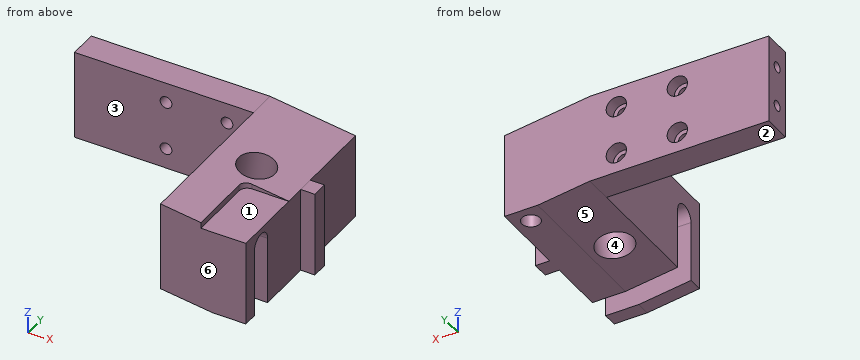
from build123d import *

# Parameters (mm, degrees)
EXTRUDE_1_DEPTH     = 23.69
CUT_EXTRUDE_1_REACH = 50.333
SKETCH_2_W          = 44
SKETCH_2_H          = 39
CUT_EXTRUDE_2_REACH = 75.348
CUT_EXTRUDE_3_DEPTH = 63.115721705
CUT_EXTRUDE_4_DEPTH = 2.79
CUT_EXTRUDE_5_REACH = 53.075
SKETCH_7_R          = 4.5
SKETCH_8_R          = 1.25
CUT_EXTRUDE_6_DEPTH = 8.5
SKETCH_10_R         = 1.45
CUT_EXTRUDE_7_DEPTH = 63.115721705
SKETCH_11_R         = 2.5
CUT_EXTRUDE_8_DEPTH = 3
SKETCH_12_R         = 2.25
CUT_EXTRUDE_9_DEPTH = 6


with BuildPart() as part:
    # 草图1 → 凸台-拉伸1 (new body)
    with BuildSketch(Plane.XY):
        Polygon((30.632183908, 5.365900383), (34.132183908, 5.365900383), (34.132183908, 1.365900383), (30.632183908, 1.365900383), (30.632183908, -21.634099617), (-34.367816092, -21.634099617), (-34.367816092, 24.365900383), (30.632183908, 24.365900383), align=None)
    extrude(amount=EXTRUDE_1_DEPTH)

    # 草图2 → 切除-拉伸1 (cut, up to next)
    with BuildSketch(Plane(origin=(0, 0, 0), x_dir=(-1, 0, 0), z_dir=(0, 0, -1)), mode=Mode.PRIVATE) as cut_extrude_1_sk1:
        with Locations((12.367816092, -2.134099617)):
            Rectangle(SKETCH_2_W, SKETCH_2_H)
    cut_extrude_1_tool1 = extrude(cut_extrude_1_sk1.sketch, amount=-CUT_EXTRUDE_1_REACH, mode=Mode.PRIVATE) & part.part
    add(cut_extrude_1_tool1.solids().sort_by_distance((-12.367816, -2.1341, 0))[0], mode=Mode.SUBTRACT)

    # 草图3 → 切除-拉伸2 (cut, up to next)
    with BuildSketch(Plane(origin=(30.632183908, 0, 0), x_dir=(0, 0, -1), z_dir=(1, 0, 0)), mode=Mode.PRIVATE) as cut_extrude_2_sk1:
        with BuildLine():
            Line((0, -18.084546462), (0, -12.484546462))
            Line((0, -12.484546462), (-16.69, -12.484546462))
            ThreePointArc((-16.69, -12.484546462), (-19.49, -15.284546462), (-16.69, -18.084546462))
            Line((-16.69, -18.084546462), (0, -18.084546462))
        make_face()
    cut_extrude_2_tool1 = extrude(cut_extrude_2_sk1.sketch, amount=-CUT_EXTRUDE_2_REACH, mode=Mode.PRIVATE) & part.part
    add(cut_extrude_2_tool1.solids().sort_by_distance((30.632184, -15.284546, 9.454896))[0], mode=Mode.SUBTRACT)

    # 草图4 → 切除-拉伸3 (cut, through all)
    with BuildSketch(Plane(origin=(0, 24.365900383, 0), x_dir=(1, 0, 0), z_dir=(0, 1, 0))):
        Polygon((9.632183908, -23.69), (34.132183908, -23.69), (34.132183908, -20.93), (30.632183908, -20.93), align=None)
        Polygon((-34.367816092, -1.69), (-34.367816092, 0), (22.482183908, 0), (9.632183908, -1.69), align=None)
    extrude(amount=-CUT_EXTRUDE_3_DEPTH, mode=Mode.SUBTRACT)

    # 草图5 → 切除-拉伸4 (cut)
    with BuildSketch(Plane.XY.offset(23.69)):
        with BuildLine():
            Line((30.632183908, -21.634099617), (19.572183908, -21.634099617))
            Line((19.572183908, -21.634099617), (19.572183908, -5.634099617))
            ThreePointArc((19.572183908, -5.634099617), (20.157970346, -4.219886054), (21.572183908, -3.634099617))
            Line((21.572183908, -3.634099617), (30.632183908, -3.634099617))
            Line((30.632183908, -3.634099617), (30.632183908, -21.634099617))
        make_face()
    extrude(amount=-CUT_EXTRUDE_4_DEPTH, mode=Mode.SUBTRACT)

    # 切除-拉伸5: up to this plane
    cut_extrude_5_end = Plane(origin=(22.482183908, -21.634099617, 0), z_dir=(0.13039463587890723, 0, 0.9914621722153636))
    # 草图7 → 切除-拉伸5 (cut, up to the surface)
    with BuildSketch(Plane(origin=(3.224230445, 0, 24.532188169), x_dir=(0.9914735684520677, 0, -0.1303079547108432), z_dir=(0.1303079547108432, 0, 0.9914735684520678)), mode=Mode.PRIVATE) as cut_extrude_5_sk1:
        with Locations((16.143060304, 2.365900383)):
            Circle(SKETCH_7_R)
    cut_extrude_5_tool1 = split(extrude(cut_extrude_5_sk1.sketch, amount=-CUT_EXTRUDE_5_REACH, mode=Mode.PRIVATE), bisect_by=cut_extrude_5_end, keep=Keep.BOTH, mode=Mode.PRIVATE)
    add(cut_extrude_5_tool1.solids().sort_by_distance((19.229648, 2.3659, 22.428619))[0], mode=Mode.SUBTRACT)

    # 草图8 → 切除-拉伸6 (cut)
    with BuildSketch(Plane.ZY.offset(34.367816092)):
        with Locations((7.69, 20.865900383)):
            Circle(SKETCH_8_R)
        with Locations((17.69, 20.865900383)):
            Circle(SKETCH_8_R)
    extrude(amount=-CUT_EXTRUDE_6_DEPTH, mode=Mode.SUBTRACT)

    # 草图10 → 切除-拉伸7 (cut, through all)
    with BuildSketch(Plane(origin=(0, 24.365900383, 0), x_dir=(1, 0, 0), z_dir=(0, 1, 0))):
        with Locations(Location((-11.867816092, -18.69, 0), (0, 0, 180))):
            Circle(SKETCH_10_R)
        with Locations(Location((-11.867816092, -6.69, 0), (0, 0, 180))):
            Circle(SKETCH_10_R)
        with Locations(Location((3.132183908, -18.69, 0), (0, 0, 180))):
            Circle(SKETCH_10_R)
        with Locations(Location((3.132183908, -6.69, 0), (0, 0, 180))):
            Circle(SKETCH_10_R)
    extrude(amount=-CUT_EXTRUDE_7_DEPTH, mode=Mode.SUBTRACT)

    # 草图11 → 切除-拉伸8 (cut)
    with BuildSketch(Plane(origin=(0, 24.365900383, 0), x_dir=(1, 0, 0), z_dir=(0, 1, 0))):
        with Locations(Location((-11.867816092, -6.69, 0), (0, 0, 180))):
            Circle(SKETCH_11_R)
        with Locations(Location((-11.867816092, -18.69, 0), (0, 0, 180))):
            Circle(SKETCH_11_R)
        with Locations(Location((3.132183908, -6.69, 0), (0, 0, 180))):
            Circle(SKETCH_11_R)
        with Locations(Location((3.132183908, -18.69, 0), (0, 0, 180))):
            Circle(SKETCH_11_R)
    extrude(amount=-CUT_EXTRUDE_8_DEPTH, mode=Mode.SUBTRACT)

    # 草图12 → 切除-拉伸9 (cut)
    with BuildSketch(Plane(origin=(0, 0, 0), x_dir=(-1, 0, 0), z_dir=(0, 0, -1))):
        with Locations((-26.632183908, 20.115900383)):
            Circle(SKETCH_12_R)
    extrude(amount=-CUT_EXTRUDE_9_DEPTH, mode=Mode.SUBTRACT)


solid = part.part
Work out the finished part from the listing and answer in its coordinate system (mm). Face numbers are marked on the shaded views. A direction names the side the tool comes from. Round coordinates to 2 decimals unless told otherwise and drop trailing zeros. Write each loop counter-clockwise with the first axis right and the second up, starting at its lowest first coordinate (ties: lowest second). Pieces come first, ordered by that corner, then holes. Notation, with made-up numbers: (58.5, 27) - (94.5, 27) arc R16 ccw to (94.5, 58) - close; hole circle Ø2 at (21.5, 0). An arc over 180 degrees is marked (long way). Answer in a Markdown table with one row per item. Add a question column.
1. A cutting plane is placed at A-A, the plane y = 10.5. Determine the outline of the cut face in (x, z), and give its area (3 significant figures).
2. A cutting plane is placed at D-D, the plane x = -16.5. Determine the outline of the cut face in (y, z), and give its area (3 significant figures).
3. A cutting plane is placed at C-C, the plane x = -28. Determine the outline of the cut face in (y, z), and give its area (3 significant figures).
4. Given pin 1 (6 mm diameter, centred on y = -12.5, z = 8.5, fed in from +X); pin 2 (5.5 mm diameter, centred on x = -3, y = 21, fed in from -Z); pin 3 (6.5 mm diameter, centred on x = -16.5, z = 17.5, fed in from -Y); pin 4 (1.7 mm diameter, centred on x = -11.87, z = 6.69, fed in from +Y), each flat-ended and moving along its own axis, determine where each tip first touches the part or whether it passes through.
5. The mould has two halves that part along X. Classify the marked faces 4, 5 and 6: +X half, -X half, draft (parallel to the pull), parting line (faces both ways), or undercut.
6. For the marked faces 1, 2 and 3, determine the directions among +Z, -Z, +X, -X, +Y, -Y from which every point of the face is accessible in a straight line to the end or side of a thin tool.
7. A cutting plane is placed at B-B, the plane x = 3. Determine the outline of the cut face in (y, z), and give its area (3 significant figures).
8. Find the intervals of material crossed by line 1 along X through (y, z) = (18.5, 18.75); line 2 along X through (y, z) = (-11, 17.25); line 3 along Y through (x, z) = (-25.5, 3.5), in increasing order. Write a range as from..to.
Worked out:
| question | item | result |
|---|---|---|
| 1 | outline | (9.63, 1.69) - (22.48, 0) - (30.63, 0) - (30.63, 20.93) - (9.63, 23.69) - close |
| 1 | area | 458 mm^2 |
| 2 | outline | (17.37, 1.69) - (24.37, 1.69) - (24.37, 23.69) - (17.37, 23.69) - close |
| 2 | area | 154 mm^2 |
| 3 | outline | (17.37, 1.69) - (24.37, 1.69) - (24.37, 23.69) - (17.37, 23.69) - close; hole circle Ø2.5 at (20.87, 7.69); hole circle Ø2.5 at (20.87, 17.69) |
| 3 | area | 144 mm^2 |
| 4 | pin 1 | x = 30.63 |
| 4 | pin 2 | z = 1.69 |
| 4 | pin 3 | y = 17.37 |
| 4 | pin 4 | through |
| 5 | face 4 | undercut |
| 5 | face 5 | -X half |
| 5 | face 6 | draft |
| 6 | face 1 | +Z, +X, -Y |
| 6 | face 2 | -Z, -X, +Y, -Y |
| 6 | face 3 | +Z, -Z, -X, -Y |
| 7 | outline | (17.37, 1.69) - (24.37, 1.69) - (24.37, 4.19) - (21.37, 4.19) - (21.37, 5.25) - (17.37, 5.25) - close; (17.37, 8.13) - (21.37, 8.13) - (21.37, 9.19) - (24.37, 9.19) - (24.37, 16.19) - (21.37, 16.19) - (21.37, 17.25) - (17.37, 17.25) - close; (17.37, 20.13) - (21.37, 20.13) - (21.37, 21.19) - (24.37, 21.19) - (24.37, 23.69) - (17.37, 23.69) - close |
| 7 | area | 101 mm^2 |
| 8 | line 1 | -34.37..-13.32, -10.42..1.68, 4.58..30.63 |
| 8 | line 2 | 9.63..30.63 |
| 8 | line 3 | 17.37..24.37 |
